Could you check a few things on this model? Use its own coordinates, in mm. Coordinates: 2 decimals unless noted, no trailing zeros. Order: outer loops, then holes, each group sorted by start corner. A loop starts at its lowest first (then second) coordinate and runs counter-clockwise, first axis right, second up. Notation, with made-up numbers: M 2,62 L 52,62 A12 cw 52,70 Z; hole C 81.5,-27 d1. An arc over 180 degrees is marked long. Write item = value, one per line. Start each with the question number.
from build123d import *

# Parameters (mm, degrees)
SKETCH1_R                    = 25
BOSS_EXTRUDE1_DEPTH          = 25
M24_TAPPED_HOLE1_D           = 21
M24_TAPPED_HOLE1_DEPTH       = 57
M24_TAPPED_HOLE1_CSINK_D     = 24.05
M24_TAPPED_HOLE1_CSINK_ANGLE = 90
M24_TAPPED_HOLE1_TIP         = 6.3090365
M8_TAPPED_HOLE1_D            = 6.8
M8_TAPPED_HOLE1_DEPTH        = 63.75
M8_TAPPED_HOLE1_CSINK_D      = 8.05
M8_TAPPED_HOLE1_CSINK_ANGLE  = 90
M8_TAPPED_HOLE1_TIP          = 2.042926105


with BuildPart() as part:
    # Sketch1 → Boss-Extrude1 (new body)
    with BuildSketch(Plane.XY):
        Circle(SKETCH1_R)
    extrude(amount=BOSS_EXTRUDE1_DEPTH)

    # M24 Tapped Hole1
    with Locations(Plane.XY.offset(25)):
        with Locations((0, 0)):
            CounterSinkHole(M24_TAPPED_HOLE1_D / 2, M24_TAPPED_HOLE1_CSINK_D / 2, depth=M24_TAPPED_HOLE1_DEPTH, counter_sink_angle=M24_TAPPED_HOLE1_CSINK_ANGLE)
            with Locations((0, 0, -(M24_TAPPED_HOLE1_DEPTH + M24_TAPPED_HOLE1_TIP / 2))):  # 118° drill point
                Cone(0, M24_TAPPED_HOLE1_D / 2, M24_TAPPED_HOLE1_TIP, mode=Mode.SUBTRACT)

    # M8 Tapped Hole1
    with Locations(Plane(origin=(-24.965469306, -1.313522862, 10.643433194), x_dir=(0.052540914496, -0.998618772257, 0), z_dir=(-0.998618772257, -0.052540914496, 0))):
        with Locations((0, 0)):
            CounterSinkHole(M8_TAPPED_HOLE1_D / 2, M8_TAPPED_HOLE1_CSINK_D / 2, depth=M8_TAPPED_HOLE1_DEPTH, counter_sink_angle=M8_TAPPED_HOLE1_CSINK_ANGLE)
            with Locations((0, 0, -(M8_TAPPED_HOLE1_DEPTH + M8_TAPPED_HOLE1_TIP / 2))):  # 118° drill point
                Cone(0, M8_TAPPED_HOLE1_D / 2, M8_TAPPED_HOLE1_TIP, mode=Mode.SUBTRACT)


solid = part.part
(1) Please list where these lines run through material, in increasing order: probe 1 along Y at (x, z) = (0, 7.75); probe 2 along X at (y, z) = (4.5, 20.5). Write a range as from..to.
(2) Thinking about a two-plate mould opening in X: for faces 1 (the flat face through (0, -11, 0)), 2 (the cylindrical face through (23.846, 7.509, 12.325)), 3 (the cylindrical face through (-10, 3.2, 11.6)), which applies, released by +X, released by -X, zero draft, split by the parting line, or undercut?
(3) Will these pins go through, and if not, where does the flat tip stop? P1, Ø2, axis at y = -19.5, z = 7, coming from the +X side; P2, Ø12, axis at x = 11.5, y = 20, coming from the -Z side; P3, Ø1.5, axis at y = 5.5, z = 10, coming from the -X side; P4, Ø5, axis at y = -14, z = 10.5, coming from the +X side.
(4) Imagine slicing it at C-C on y = 0. Give the number of separate pieces and of enclosed holes in the cut face, plus the area to 3 significant figures.
(5) Imagine slicing it at D-D on y = -22. List the corners of the cut face in (x, z) for me.
(6) Imagine slicing it at A-A on x = 0. List the corners of the cut face in (y, z) for me (3 decimals).
(7) Imagine slicing it at B-B on z = 15.5. List the corners of the cut face in (x, y) for me, plus the area to 3 significant figures.
Response:
q1.probe_1 = -25..-10.5, 10.5..25
q1.probe_2 = -24.59..-9.49, 9.49..24.59
q2.face_1 = zero draft
q2.face_2 = split by the parting line
q2.face_3 = undercut
q3.P1 = 16.82
q3.P2 = 0
q3.P3 = -24.54
q3.P4 = 22.2
q4.separate_pieces = 4
q4.enclosed_holes = 0
q4.area = 533 mm2
q5.outline = M -11.87,0 L 11.87,0 L 11.87,25 L -11.87,25 Z
q6.outline = M -25,0 L -10.5,0 L -10.5,23.475 L -12.025,25 L -25,25 Z; M 10.5,0 L 25,0 L 25,25 L 12.025,25 L 10.5,23.475 Z
q7.outline = C 0,0 d50; hole C 0,0 d21
q7.area = 1,620 mm2
